Print and shaded views of the part. All mm, measured from the part's lowest x, y and z. Round coordinates to 2 decimals unless told otherwise and drop trailing zeros. Loops run counter-clockwise (first coordinate to the right, second up) from the corner with the lowest first, then second, coordinate; pieces in that order, holes last. Notation, with made-up numbers: (13.5, 62.5) - (66.5, 62.5) arc R20 cw to (66.5, 86.5) - close; hole circle Ø8 at (56.25, -16). An arc over 180 degrees is marked (long way). Answer as a JSON object with one key per item and string values.
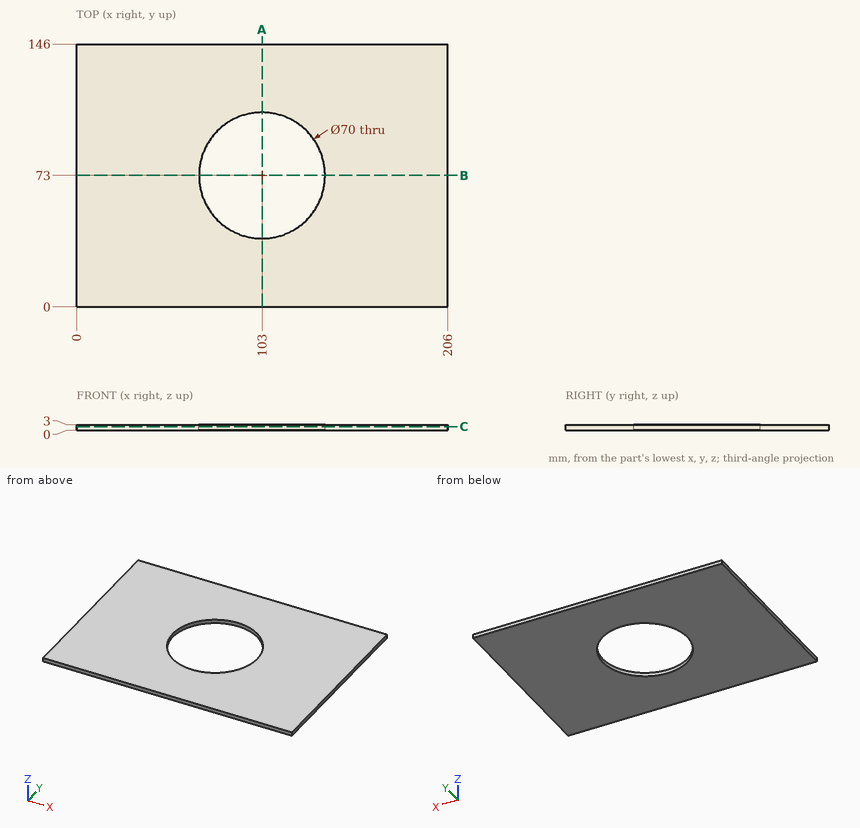
1) Slice it at B-B on y = 73. List the corners of the cut face in (x, z), then the cut area to 3 significant figures.
Values follow:
{"outline": "(0, 0) - (68, 0) - (68, 3) - (0, 3) - close; (138, 0) - (206, 0) - (206, 3) - (138, 3) - close", "area": "408 mm²"}
2) Slice it at C-C on z = 2.05. List the corners of the cut face in (x, y), then the cut area to 3 significant figures.
Values follow:
{"outline": "(0, 0) - (206, 0) - (206, 146) - (0, 146) - close; hole circle Ø70 at (103, 73)", "area": "26,200 mm²"}
3) Probe probe 1 along Y at (x, z) = (103, 1.5); probe 2 along X at (y, z) = (97.5, 0.35) (3 decimals); probe 3 along X at (y, z) = (97, 1.8). List the from-to ranges inside material, lowest first.
Values follow:
{"probe 1": "0 to 38, 108 to 146", "probe 2": "0 to 78.005, 127.995 to 206", "probe 3": "0 to 77.52, 128.48 to 206"}
4) Slice it at A-A on x = 103. List the corners of the cut face in (y, z), then the cut area to 3 significant figures.
Values follow:
{"outline": "(0, 0) - (38, 0) - (38, 3) - (0, 3) - close; (108, 0) - (146, 0) - (146, 3) - (108, 3) - close", "area": "228 mm²"}
